For this review, take the finished solid that the model builds, in its own axes (mm). Coordinates: 2 decimals unless noted, no trailing zeros. Order: outer loops, then holes, each group sorted by start corner. A loop starts at its lowest first (then second) coordinate and runs counter-clockwise, first axis right, second up. Notation, with made-up numbers: (53, 11) -> (72, 11) arc R23 cw to (72, 19) -> close; hole circle Ø1 at (3, 61.5). An arc over 180 degrees is marked (long way). Return JSON: item names as keys, results as strings. Group by question number.
Item 1: Take a section at D-D (y = 45). Write out the cut boundary in (x, z).
Item 2: Insertion check: pin 1 (5 mm diameter, centred on y = 12.5, z = 14.5, fed in from +X); pin 2 (12 mm diameter, centred on y = -38.5, z = 16.5, fed in from +X). Each pin has a flat end and moves straight along its axis. Give the tip position at first contact, or say it passes through.
Item 3: For line 1 along X through (y, z) = (-15, 17); line 2 along Y through (x, z) = (-250, 6.75); line 3 along Y through (x, z) = (250, 8.25), list the stretches that pass through material, from the lowest coordinate up.
Item 4: Take a section at C-C (y = -44.5). Write out the cut boundary in (x, z), then the cut area to 3 significant figures.
Item 5: Take a section at A-A (y = 0). Write out the cut boundary in (x, z), then the cut area to 3 significant figures.
Item 6: Take a section at B-B (z = 16.75). Write out the cut boundary in (x, y).
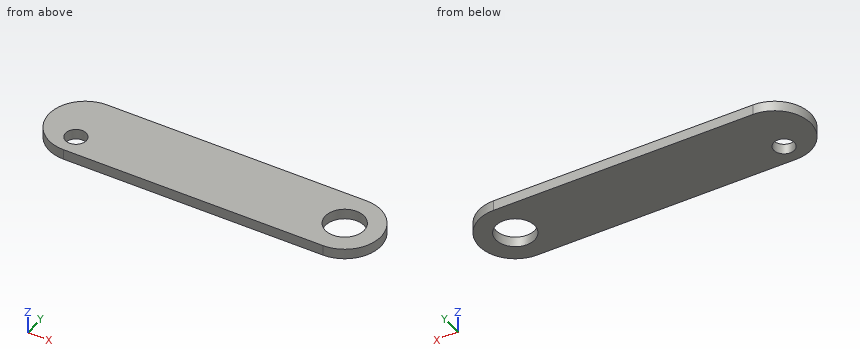
```python
from build123d import *

# Parameters (mm, degrees)
SKETCH_1_R      = 37.5
SKETCH_1_R_2    = 20
EXTRUDE_1_DEPTH = 20


with BuildPart() as part:
    # 草图1 → 凸台-拉伸1 (new body)
    with BuildSketch(Plane.XY):
        with BuildLine():
            Line((-250, 70), (250, 70))
            ThreePointArc((250, 70), (320, 0), (250, -70))
            Line((250, -70), (-250, -70))
            ThreePointArc((-250, -70), (-320, 0), (-250, 70))
        make_face()
        with Locations((250, 0)):
            Circle(SKETCH_1_R, mode=Mode.SUBTRACT)
        with Locations((-250, -30)):
            Circle(SKETCH_1_R_2, mode=Mode.SUBTRACT)
    extrude(amount=EXTRUDE_1_DEPTH)


solid = part.part
```
Findings below:
{
 "1": {"outline": "(-303.62, 0) -> (303.62, 0) -> (303.62, 20) -> (-303.62, 20) -> close"},
 "2": {"pin 1": "stops at x = 319.28", "pin 2": "stops at x = 312"},
 "3": {"line 1": "x = -318.37 to -263.23, -236.77 to 215.63, 284.37 to 318.37", "line 2": "y = -70 to -50, -10 to 70", "line 3": "y = -70 to -37.5, 37.5 to 70"},
 "4": {"outline": "(-304.03, 0) -> (-263.77, 0) -> (-263.77, 20) -> (-304.03, 20) -> close; (-236.23, 0) -> (304.03, 0) -> (304.03, 20) -> (-236.23, 20) -> close", "area": "11,600 mm2"},
 "5": {"outline": "(-320, 0) -> (212.5, 0) -> (212.5, 20) -> (-320, 20) -> close; (287.5, 0) -> (320, 0) -> (320, 20) -> (287.5, 20) -> close", "area": "11,300 mm2"},
 "6": {"outline": "(-250, -70) -> (250, -70) arc R70 ccw to (250, 70) -> (-250, 70) arc R70 ccw to start; hole circle Ø40 at (-250, -30); hole circle Ø75 at (250, 0)"}
}
